Source: CAD feature listing. Evaluate the final solid. Frame: model axes, mm. Face numbers are marked on the shaded views. A direction names the side the tool comes from. Round coordinates to 2 decimals unless told otherwise and drop trailing zeros. Loops run counter-clockwise (first coordinate to the right, second up) from the corner with the lowest first, then second, coordinate; pieces in that order, holes last. Notation, with made-up numbers: (75.25, -25.75) -> (133.25, -25.75) arc R22 ccw to (133.25, -16.75) -> close; hole circle Ø7 at (-37.5, -25.5). An arc over 180 degrees is marked (long way). Return JSON: item names as keys, results as strings. Group by question number.
```python
from build123d import *

# Parameters (mm, degrees)
BASE_DISC_SKETCH_R        = 31
BASE_DISC_62_DEPTH        = 13
RELIEF_CUT_SKETCH_R       = 10
RELIEF_CUT_DEPTH          = 46.727453461
THREE_ARM_BOSS_DEPTH      = 19
ARM_GAP_SKETCH_R          = 2.5
ARM_GAP_CUT_DEPTH         = 48.780749262
RADIAL_HOLE_SKETCH_R      = 5
RADIAL_HOLE_10_DEPTH      = 5
ARM_CUTS_PATTERN_3X_COUNT = 3
ARM_CHAMFERS_5MM_SIZE     = 5


with BuildPart() as part:
    # Base Disc Sketch → Base Disc Ø62 (new body)
    with BuildSketch(Plane.XY):
        with Locations(Location((0, 0, 0), (0, 0, 180))):
            Circle(BASE_DISC_SKETCH_R)
    extrude(amount=BASE_DISC_62_DEPTH)

    # Relief Cut Sketch → Relief Cut (cut, through all)
    with BuildSketch(Plane.XY.offset(13)):
        Circle(RELIEF_CUT_SKETCH_R)
    extrude(amount=-RELIEF_CUT_DEPTH, mode=Mode.SUBTRACT)

    # Arms Profile Sketch → Three-Arm Boss (add)
    with BuildSketch(Plane.XY.offset(13)):
        with BuildLine():
            Line((-5, 8.660254038), (-5, 30.594117082))
            ThreePointArc((-5, 30.594117082), (-7.526051267, 30.072554802), (-10, 29.342801502))
            Line((-10, 29.342801502), (-10, 8.660254038))
            ThreePointArc((-10, 8.660254038), (-10.669872981, 6.160254038), (-12.5, 4.330127019))
            Line((-12.5, 4.330127019), (-30.411611519, -6.011146713))
            ThreePointArc((-30.411611519, -6.011146713), (-29.806622049, -8.518525814), (-28.995282599, -10.966931522))
            Line((-28.995282599, -10.966931522), (-10, 0))
            ThreePointArc((-10, 0), (-8.660254038, 5), (-5, 8.660254038))
        make_face()
        with BuildLine():
            ThreePointArc((12.5, 4.330127019), (10.669872981, 6.160254038), (10, 8.660254038))
            Line((10, 8.660254038), (10, 29.342801502))
            ThreePointArc((10, 29.342801502), (7.526051267, 30.072554802), (5, 30.594117082))
            Line((5, 30.594117082), (5, 8.660254038))
            ThreePointArc((5, 8.660254038), (8.660254038, 5), (10, 0))
            Line((10, 0), (28.995282599, -10.966931522))
            ThreePointArc((28.995282599, -10.966931522), (29.806622049, -8.518525814), (30.411611519, -6.011146713))
            Line((30.411611519, -6.011146713), (12.5, 4.330127019))
        make_face()
        with BuildLine():
            ThreePointArc((20.411611519, -23.331654789), (22.280570782, -21.554028988), (23.995282599, -19.62718556))
            Line((23.995282599, -19.62718556), (5, -8.660254038))
            ThreePointArc((5, -8.660254038), (0, -10), (-5, -8.660254038))
            Line((-5, -8.660254038), (-23.995282599, -19.62718556))
            ThreePointArc((-23.995282599, -19.62718556), (-22.280570782, -21.554028988), (-20.411611519, -23.331654789))
            Line((-20.411611519, -23.331654789), (-2.5, -12.990381057))
            ThreePointArc((-2.5, -12.990381057), (0, -12.320508076), (2.5, -12.990381057))
            Line((2.5, -12.990381057), (20.411611519, -23.331654789))
        make_face()
    extrude(amount=THREE_ARM_BOSS_DEPTH)

    # Arm Gap Sketch → Arm Gap Cut (cut, through all)
    with BuildSketch(Plane.XY.offset(13)):
        with Locations((-6.470476128, -24.148145657)):
            Circle(ARM_GAP_SKETCH_R)
    arm_gap_cut = extrude(amount=-ARM_GAP_CUT_DEPTH, mode=Mode.SUBTRACT)

    # Radial Hole Sketch → Radial Hole Ø10 (cut)
    with BuildSketch(Plane.XY.offset(13)):
        with Locations((-6.470476128, -24.148145657)):
            Circle(RADIAL_HOLE_SKETCH_R)
    radial_hole_10 = extrude(amount=-RADIAL_HOLE_10_DEPTH, mode=Mode.SUBTRACT)

    # Arm Cuts Pattern 3x: Arm Gap Cut, Radial Hole Ø10 ×3 about axis
    arm_cuts_pattern_3x_axis = Axis((0, 0, 0), (0, 0, 1))
    add([arm_gap_cut.rotate(arm_cuts_pattern_3x_axis, i * 360 / ARM_CUTS_PATTERN_3X_COUNT) for i in range(1, ARM_CUTS_PATTERN_3X_COUNT)], mode=Mode.SUBTRACT)
    add([radial_hole_10.rotate(arm_cuts_pattern_3x_axis, i * 360 / ARM_CUTS_PATTERN_3X_COUNT) for i in range(1, ARM_CUTS_PATTERN_3X_COUNT)], mode=Mode.SUBTRACT)

    # Arm Chamfers 5mm
    arm_chamfers_5mm_edges = [part.edges().sort_by_distance(p)[0] for p in [
        (-29.806622049, -8.518525814, 32),
        (-7.526051267, 30.072554802, 32),
        (7.526051267, 30.072554802, 32),
        (29.806622049, -8.518525814, 32),
        (22.280570782, -21.554028988, 32),
        (-22.280570782, -21.554028988, 32),
    ]]
    chamfer(arm_chamfers_5mm_edges, length=ARM_CHAMFERS_5MM_SIZE)


solid = part.part
```
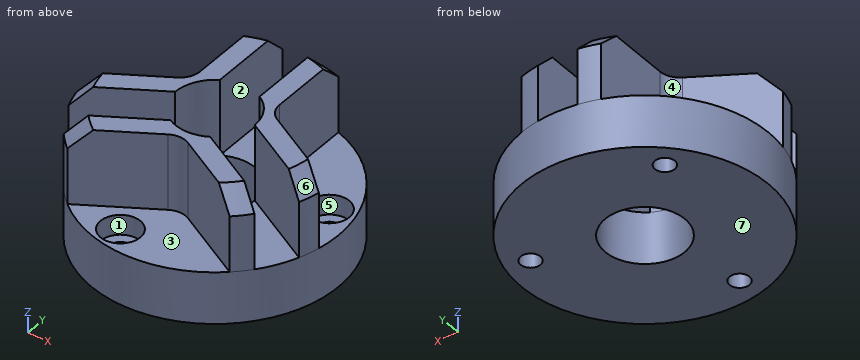
(1) Set-up query: the marked faces 1, 2, 3 and 4. Return all of +Z, -Z, +X, -X, +Y, -Y with unobstructed straight access to the full face (end or side cutting, diameter ignored); none if empty.
(2) Ray query, line 1 (X direction, y = 21.5, z = 17); line 2 (Z direction, x = 16, y = -24); line 3 (Y direction, x = 2, z = 12.5). Return the intervals inside material, ascending.
(3) Cut plane C-C (y = 7). Return loops of the section in (x, z), and give its area (3 significant figures).
(4) Mould query, pull axis Y, two halves, no side actions, for the marked faces 5, 6 and 7. Classes: released by +Y, released by -Y, zero draft, split by the parting line, or undercut.
(5) Cut plane B-B (z = 18). Return loops of the section in (x, y), and give its area (3 significant figures).
(6) Cut plane A-A (x = 0). Return loops of the section in (y, z), and give its area (3 significant figures).
(7) Pin query (flat end, axial travel): pin 1 (6 mm diameter, centred on x = 18, y = -10.5, fed in from +Z); pin 2 (6 mm diameter, centred on x = 24.15, y = 6.47, fed in from +Z); pin 3 (4 mm diameter, centred on x = -15, z = 17, fed in from +Y). Return the tip coordinate at first contact, or that it passes through.
(8) Cut plane D-D (y = -14). Return loops of the section in (x, z), and give its area (3 significant figures).
Answers follow:
{
 "1": {"face 1": "+Z", "face 2": "+Z, +Y", "face 3": "+Z, -Y", "face 4": "+Z, -X, +Y"},
 "2": {"line 1": "-10 to -5, 5 to 10", "line 2": "0 to 13", "line 3": "-30.94 to -9.8, 9.8 to 30.94"},
 "3": {"outline": "(-30.2, 0) -> (-7.14, 0) -> (-7.14, 32) -> (-10.28, 32) -> (-10.28, 13) -> (-30.2, 13) -> close; (7.14, 0) -> (21.7, 0) -> (21.7, 8) -> (19.18, 8) -> (19.18, 13) -> (10.28, 13) -> (10.28, 32) -> (7.14, 32) -> close; (26.59, 0) -> (30.2, 0) -> (30.2, 13) -> (29.12, 13) -> (29.12, 8) -> (26.59, 8) -> close", "area": "630 mm^2"},
 "4": {"face 5": "undercut", "face 6": "released by -Y", "face 7": "zero draft"},
 "5": {"outline": "(-30.41, -6.01) arc R31 ccw to (-29, -10.97) -> (-10, 0) arc R10 cw to (-5, 8.66) -> (-5, 30.59) arc R31 ccw to (-10, 29.34) -> (-10, 8.66) arc R5 cw to (-12.5, 4.33) -> close; (-24, -19.63) arc R31 ccw to (-20.41, -23.33) -> (-2.5, -12.99) arc R5 cw to (2.5, -12.99) -> (20.41, -23.33) arc R31 ccw to (24, -19.63) -> (5, -8.66) arc R10 cw to (-5, -8.66) -> close; (5, 8.66) arc R10 cw to (10, 0) -> (29, -10.97) arc R31 ccw to (30.41, -6.01) -> (12.5, 4.33) arc R5 cw to (10, 8.66) -> (10, 29.34) arc R31 ccw to (5, 30.59) -> close", "area": "705 mm^2"},
 "6": {"outline": "(-31, 0) -> (-10, 0) -> (-10, 32) -> (-12.32, 32) -> (-12.32, 13) -> (-31, 13) -> close; (10, 0) -> (31, 0) -> (31, 13) -> (10, 13) -> close", "area": "590 mm^2"},
 "7": {"pin 1": "z = 13", "pin 2": "z = 8", "pin 3": "y = 4.04"},
 "8": {"outline": "(-27.66, 0) -> (27.66, 0) -> (27.66, 13) -> (14.25, 13) -> (14.25, 32) -> (4.25, 32) -> (4.25, 13) -> (-4.25, 13) -> (-4.25, 32) -> (-14.25, 32) -> (-14.25, 13) -> (-27.66, 13) -> close", "area": "1,100 mm^2"}
}
